Can you work these out from the model? Positions are in its coordinate system, mm. Face numbers are marked on the shaded views. A direction names the side the tool comes from. Round coordinates to 2 decimals unless told otherwise and drop trailing zeros. Order: outer loops, then holes, each group sorted by start corner. A loop starts at its lowest first (then second) coordinate and runs counter-clockwise, first axis right, second up.
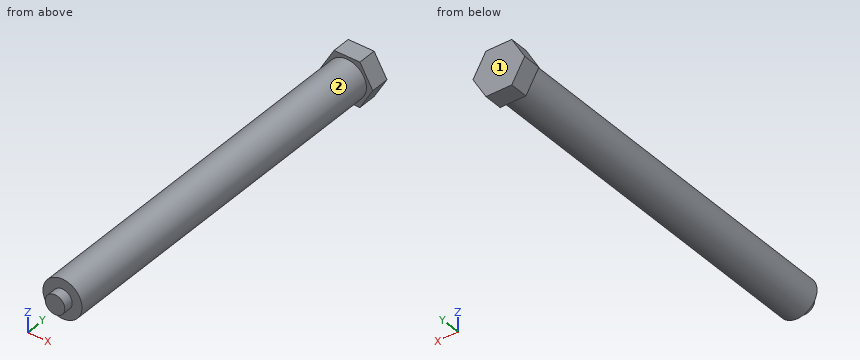
from build123d import *

# Parameters (mm, degrees)
SKETCH2_OUTSIDE_W  = 138.358
SKETCH2_OUTSIDE_H  = 138.358
CUT_EXTRUDE1_DEPTH = 32


with BuildPart() as part:
    # Sketch1 → Revolve1 (revolve)
    with BuildSketch(Plane.XY, mode=Mode.PRIVATE) as revolve1_sk:
        Polygon((0, 0), (10, 0), (10, 10), (20, 10), (20, 391), (26.5, 391), (26.5, 410), (0, 410), align=None)
    revolve(revolve1_sk.sketch.rotate(Axis((0, 0, 0), (0, 1, 0)), 90), axis=Axis((0, 0, 0), (0, 1, 0)))

    # Sketch2 outside → Cut-Extrude1 (cut)
    with BuildSketch(Plane(origin=(0, 410, 0), x_dir=(1, 0, 0), z_dir=(0, 1, 0))):
        Rectangle(SKETCH2_OUTSIDE_W, SKETCH2_OUTSIDE_H)
        Polygon((-26.5, 0), (-13.25, -22.9496732), (13.25, -22.9496732), (26.5, 0), (13.25, 22.9496732), (-13.25, 22.9496732), align=None, mode=Mode.SUBTRACT)
    extrude(amount=-CUT_EXTRUDE1_DEPTH, mode=Mode.SUBTRACT)


solid = part.part
(1) I want a section at B-B, the plane z = 6. List the corners of the cut face in (x, y) for me, plus the area to 3 significant figures.
(2) I want a section at C-C, the plane y = 324.5. List the corners of the cut face in (x, z) for me, plus the area to 3 significant figures.
(3) On a 3-axis mill with a long thin cutter (end or side, diameter ignored), from which of +Z, -Z, +X, -X, +Y, -Y can I reach the whole of each face in a straight line? I mean the marked faces 1 and 2. Say none if no direction works.
(4) I'm going to push flat-ended pins straight in: pin 1 Ø1.5 at (x, z) = (-19.5, 0.5) entering from -Y; pin 2 Ø3 at (y, z) = (362, -3.5) entering from +X; pin 3 Ø1.5 at (y, z) = (143, 8) entering from +X; pin 4 Ø20 at (x, z) = (3, 8) entering from -Y. Where does each tip first touch, or does it pass through?
(5) I want a section at D-D, the plane z = -14.5. List the corners of the cut face in (x, y) for me.
(6) I want a section at A-A, the plane x = 0. List the corners of the cut face in (y, z) for me.
(7) Please list where these lines run through material, in increasing order: probe 1 along Y at (x, z) = (10, 11); probe 2 along Z at (x, y) = (-15, 305); probe 3 along Y at (x, z) = (-18, 14).
Ans:
1. outline: (-23.04, 391) - (-19.08, 391) - (-19.08, 10) - (-8, 10) - (-8, 0) - (8, 0) - (8, 10) - (19.08, 10) - (19.08, 391) - (23.04, 391) - (23.04, 410) - (-23.04, 410) - close
1. area: 15,600 mm2
2. outline: circle Ø40 at (0, 0)
2. area: 1,260 mm2
3. face 1: +Z, -Z, +X, -X, +Y
3. face 2: -Y
4. pin 1: stops at y = 10
4. pin 2: stops at x = 19.9
4. pin 3: stops at x = 18.64
4. pin 4: stops at y = 0
5. outline: (-18.13, 391) - (-13.77, 391) - (-13.77, 10) - (13.77, 10) - (13.77, 391) - (18.13, 391) - (18.13, 410) - (-18.13, 410) - close
6. outline: (0, -10) - (10, -10) - (10, -20) - (391, -20) - (391, -22.95) - (410, -22.95) - (410, 22.95) - (391, 22.95) - (391, 20) - (10, 20) - (10, 10) - (0, 10) - close
7. probe 1: y = 10 to 410
7. probe 2: z = -13.23 to 13.23
7. probe 3: y = 391 to 410
